Geometry: final body of the model. Coordinates: model frame, mm. Face numbers are marked on the shaded views. A direction names the side the tool comes from. Round coordinates to 2 decimals unless told otherwise and drop trailing zeros. Loops run counter-clockwise (first coordinate to the right, second up) from the corner with the lowest first, then second, coordinate; pieces in that order, holes last. Notation, with made-up numbers: M 68,87 L 74,87 A17 ccw 74,112 Z; hole C 14.25,18 d7. An arc over 180 degrees is marked long. Answer as a JSON object with one key per item and string values.
from build123d import *

# Parameters (mm, degrees)
EXTRUDE_1_DEPTH     = 150
CUT_EXTRUDE_1_DEPTH = 150
CUT_EXTRUDE_2_DEPTH = 150


with BuildPart() as part:
    # 草图1 → 凸台-拉伸1 (new body)
    with BuildSketch(Plane.XY):
        with BuildLine():
            Line((0, 0), (0, -56))
            ThreePointArc((0, -56), (2.928932188, -63.071067812), (10, -66))
            Line((10, -66), (355, -66))
            Line((355, -66), (355, -58))
            Line((355, -58), (10, -58))
            ThreePointArc((10, -58), (8.585786438, -57.414213562), (8, -56))
            Line((8, -56), (8, 0))
            Line((8, 0), (0, 0))
        make_face()
    extrude(amount=EXTRUDE_1_DEPTH)

    # 草图2 → 切除-拉伸1 (cut)
    with BuildSketch(Plane.ZY):
        with BuildLine():
            Line((26.5, -26), (26.5, -33))
            ThreePointArc((26.5, -33), (20, -39.5), (13.5, -33))
            Line((13.5, -33), (13.5, -26))
            ThreePointArc((13.5, -26), (20, -19.5), (26.5, -26))
        make_face()
        with BuildLine():
            Line((81.5, -26), (81.5, -33))
            ThreePointArc((81.5, -33), (75, -39.5), (68.5, -33))
            Line((68.5, -33), (68.5, -26))
            ThreePointArc((68.5, -26), (75, -19.5), (81.5, -26))
        make_face()
        with BuildLine():
            Line((136.5, -26), (136.5, -33))
            ThreePointArc((136.5, -33), (130, -39.5), (123.5, -33))
            Line((123.5, -33), (123.5, -26))
            ThreePointArc((123.5, -26), (130, -19.5), (136.5, -26))
        make_face()
    extrude(amount=-CUT_EXTRUDE_1_DEPTH, mode=Mode.SUBTRACT)

    # 草图3 → 切除-拉伸2 (cut)
    with BuildSketch(Plane(origin=(0, -58, 0), x_dir=(1, 0, 0), z_dir=(0, 1, 0))):
        with BuildLine():
            Line((310, -16), (335, -16))
            ThreePointArc((335, -16), (344, -25), (335, -34))
            Line((335, -34), (310, -34))
            ThreePointArc((310, -34), (301, -25), (310, -16))
        make_face()
        with BuildLine():
            Line((310, -66), (335, -66))
            ThreePointArc((335, -66), (344, -75), (335, -84))
            Line((335, -84), (310, -84))
            ThreePointArc((310, -84), (301, -75), (310, -66))
        make_face()
        with BuildLine():
            Line((310, -116), (335, -116))
            ThreePointArc((335, -116), (344, -125), (335, -134))
            Line((335, -134), (310, -134))
            ThreePointArc((310, -134), (301, -125), (310, -116))
        make_face()
    extrude(amount=-CUT_EXTRUDE_2_DEPTH, mode=Mode.SUBTRACT)


solid = part.part
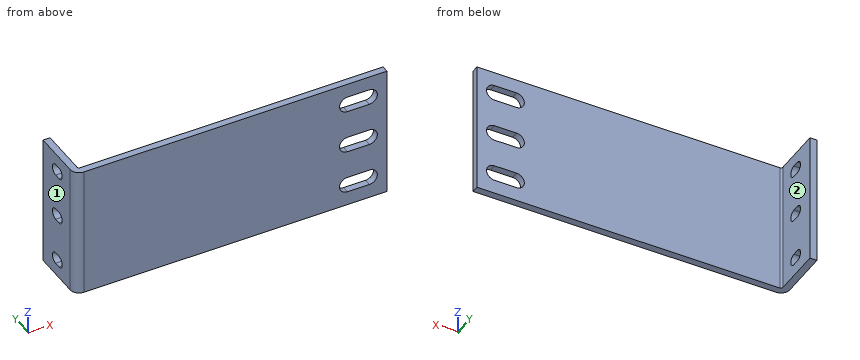
1) Section query A-A (z = 75). Return the cut outline in (x, y), and give its area (3 significant figures).
Results:
{"outline": "M 0,-56 A10 ccw 10,-66 L 301,-66 L 301,-58 L 10,-58 A2 cw 8,-56 L 8,-39.5 L 0,-39.5 Z; M 0,-19.5 L 8,-19.5 L 8,0 L 0,0 Z; M 344,-66 L 355,-66 L 355,-58 L 344,-58 Z", "area": "2,780 mm2"}
2) Reachability of the marked faces 1 and 2 from +Z, -Z, +X, -X, +Y, -Y: full face, straight path, thin tool, end or side. Return the list, or none.
Results:
{"face 1": "+Z, -Z, -X, +Y, -Y", "face 2": "+Z, -Z, +X, +Y"}
3) Section query B-B (z = 44). Return the cut outline in (x, y).
Results:
{"outline": "M 0,-56 A10 ccw 10,-66 L 355,-66 L 355,-58 L 10,-58 A2 cw 8,-56 L 8,0 L 0,0 Z"}
4) Section query D-D (x = 197.5). Return the cut outline in (y, z), and give its area (3 significant figures).
Results:
{"outline": "M -66,0 L -58,0 L -58,150 L -66,150 Z", "area": "1,200 mm2"}
5) Ray query, line 1 (Z direction, x = 317, y = -58.5); line 2 (Y direction, x = 252, z = 143); line 3 (X direction, y = -23, z = 42). Return the intervals inside material, ascending.
Results:
{"line 1": "0 to 16, 34 to 66, 84 to 116, 134 to 150", "line 2": "-66 to -58", "line 3": "0 to 8"}
6) Section query C-C (y = -46.5). Return the cut outline in (x, z).
Results:
{"outline": "M 0,0 L 8,0 L 8,150 L 0,150 Z"}
7) Pin query (flat end, axial travel): P1, Ø4, axis at x = 157, z = 40.5, coming from the +Y side; P2, Ø4, axis at x = 328.5, y = -61, coming from the -Z side; P3, Ø12, axis at y = -20.5, z = 49, coming from the +X side. Return the tip coordinate at first contact, or that it passes through.
Results:
{"P1": "y = -58", "P2": "z = 0", "P3": "x = 8"}
